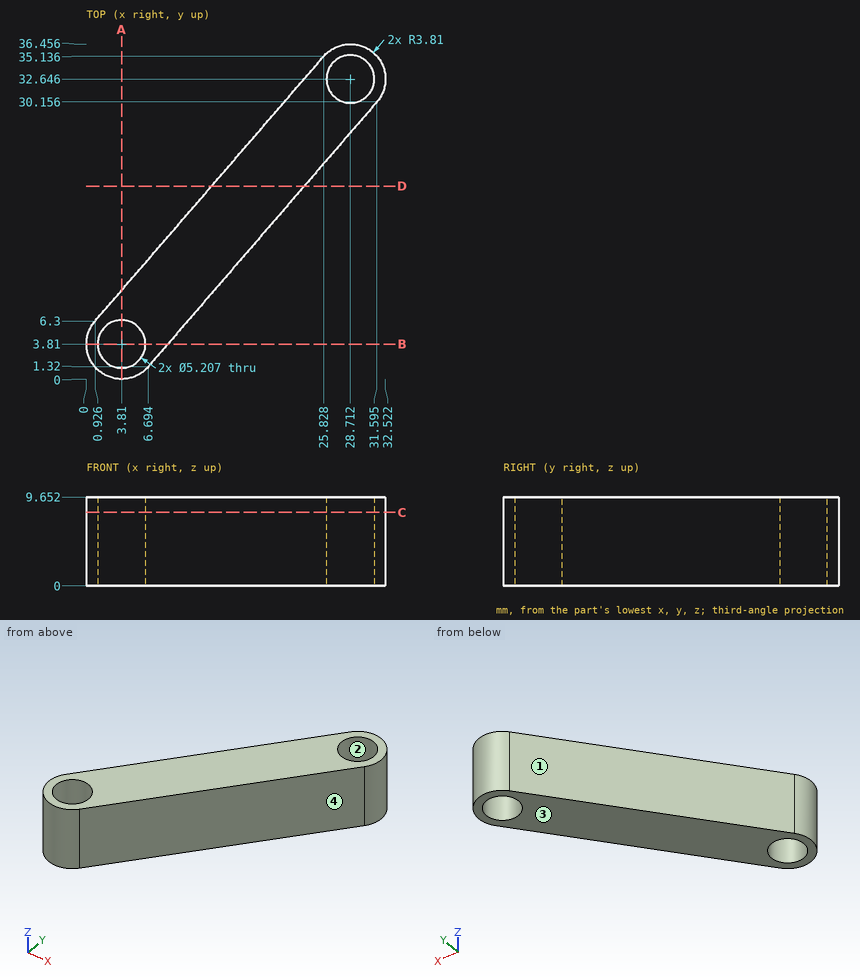
Here's the drawing with two shaded views (mm, measured from the low corner). I have some questions. Coordinates: 2 decimals unless noted, no trailing zeros. Order: outer loops, then holes, each group sorted by start corner. A loop starts at its lowest first (then second) coordinate and runs counter-clockwise, first axis right, second up.
Item 1: If we mould it in two halves opening along Y, with no side actions, what happens to the marked faces 1, 2, 3 and 4? For each: +Y half, -Y half, draft (parallel to the pull), parting line (faces both ways), or undercut.
Result sheet:
face 1: +Y half
face 2: undercut
face 3: draft
face 4: -Y half
Item 2: If we section it at C-C on z = 8: State how many separate pieces and enclosed holes the cut face has, plus the area to 3 significant figures.
Result sheet:
separate pieces: 1
enclosed holes: 2
area: 293 mm2
Item 3: If we section it at D-D on y = 21: List the corners of the cut face in (x, z) for me.
Result sheet:
outline: (13.62, 0) - (23.69, 0) - (23.69, 9.65) - (13.62, 9.65) - close
Item 4: If we section it at A-A on x = 3.81: List the corners of the cut face in (y, z) for me.
Result sheet:
outline: (0, 0) - (1.21, 0) - (1.21, 9.65) - (0, 9.65) - close; (6.41, 0) - (9.64, 0) - (9.64, 9.65) - (6.41, 9.65) - close
Item 5: For P1, Ø1, axis at y = 12.5, z = 5.5, coming from the -X side; P2, Ø3, axis at x = 3.81, y = 3.81, coming from the +Z side; P3, Ø1.5, axis at y = 11.5, z = 6, coming from the +X side; P4, Ø4, axis at x = 18.5, z = 3.5, coming from the +Y side (1 decimal), each with a flat end and sliding along its axis, tell me the tip position at first contact or that it passes through.
Result sheet:
P1: stops at x = 5.85
P2: passes through
P3: stops at x = 16.13
P4: stops at y = 29
Item 6: I need wall thicknesses on line 1 (Y direction, x = 3.81, z = 2.75) (1 decimal); line 2 (X direction, y = 3.81, z = 2) (1 decimal); line 3 (X direction, y = 4, z = 0.5) (1 decimal). Which ranges of each line are inside material? Lowest first, please.
Result sheet:
line 1: y = 0 to 1.2, 6.4 to 9.6
line 2: x = 0 to 1.2, 6.4 to 8.8
line 3: x = 0 to 1.2, 6.4 to 9
Item 7: If we section it at B-B on y = 3.81: List the corners of the cut face in (x, z) for me.
Result sheet:
outline: (0, 0) - (1.21, 0) - (1.21, 9.65) - (0, 9.65) - close; (6.41, 0) - (8.84, 0) - (8.84, 9.65) - (6.41, 9.65) - close
